Verification items for the finished model (mm, model axes). Face numbers are marked on the shaded views. A direction names the side the tool comes from. Give positions to 0.01 mm unless a question says otherwise; leave off trailing zeros. Loops run counter-clockwise (first coordinate to the right, second up) from the corner with the lowest first, then second, coordinate; pieces in that order, holes last. Notation, with made-up numbers: (72, 56.5) -> (131, 56.5) arc R33 ccw to (131, 91.5) -> close; hole circle Ø7 at (85, -12). An arc over 180 degrees is marked (long way). Answer in a Markdown table with one row per item. Add a question column.
Q1. Set-up check for the marked faces 1 and 2: record each of +Z, -Z, +X, -X, +Y, -Y from which the full face is reachable in a straight line by a thin tool's end or side.
Q2. Section check A-A on y = 3.5. Enter the section's corners in (x, z).
Q3. Gauge pin test, flat ends, axial feed: P1, Ø3, axis at x = 19, z = -11.5, coming from the +Y side; P2, Ø2, axis at x = 19, z = 6.5, coming from the -Y side (3 decimals); P3, Ø2, axis at x = 20, y = -6.5, coming from the -Z side (3 decimals). Record the tip position at first contact, or that the pin passes through.
Q4. Section check C-C on x = 17. Enter the section's corners in (y, z), and give its area (3 significant figures).
Q5. Section check B-B on z = -4. Enter the section's corners in (x, y).
Q6. Section check D-D on z = -13.5. Enter the section's corners in (x, y).
Q7. Material ranges on probe 1 along Y at (x, z) = (15, 0); probe 2 along Y at (x, z) = (18.25, 7); probe 3 along Z at (x, y) = (17.75, -7.5), recorded low to high.
Q8. Release check for a two-part mould opening along Y. For the marked faces 3, 4 and 5 record: pulls with the +Y half, pulls with the -Y half, needs draft (parallel to the pull), parting line crosses it, or undercut.
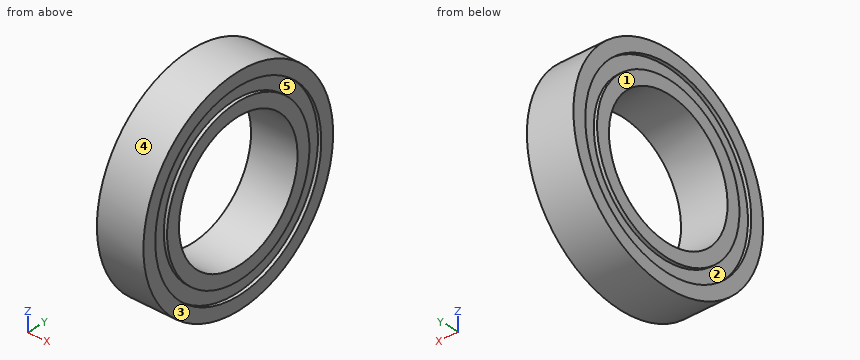
```python
from build123d import *


with BuildPart() as part:
    # Sketch1 → Revolve1 (revolve)
    with BuildSketch(Plane.XY, mode=Mode.PRIVATE) as revolve1_sk:
        Polygon((14.644406169, 14), (14.644406169, 16), (21.644406169, 16), (21.644406169, 14), (21.144406169, 14), (21.144406169, 12), (21.644406169, 12), (21.644406169, 10), (14.644406169, 10), (14.644406169, 12), (15.144406169, 12), (15.144406169, 14), align=None)
    revolve(revolve1_sk.sketch.rotate(Axis((0, 0, 0), (1, 0, 0)), 90), axis=Axis((0, 0, 0), (1, 0, 0)))


solid = part.part
```
Taken from the geometry:
| question | item | result |
|---|---|---|
| 1 | face 1 | +Z, -Z, -X, +Y, -Y |
| 1 | face 2 | -X |
| 2 | outline | (14.64, -15.61) -> (21.64, -15.61) -> (21.64, -13.56) -> (21.14, -13.56) -> (21.14, -11.48) -> (21.64, -11.48) -> (21.64, -9.37) -> (14.64, -9.37) -> (14.64, -11.48) -> (15.14, -11.48) -> (15.14, -13.56) -> (14.64, -13.56) -> close; (14.64, 9.37) -> (21.64, 9.37) -> (21.64, 11.48) -> (21.14, 11.48) -> (21.14, 13.56) -> (21.64, 13.56) -> (21.64, 15.61) -> (14.64, 15.61) -> (14.64, 13.56) -> (15.14, 13.56) -> (15.14, 11.48) -> (14.64, 11.48) -> close |
| 3 | P1 | stops at y = 12.49 |
| 3 | P2 | stops at y = -15.025 |
| 3 | P3 | stops at z = -15.025 |
| 4 | outline | circle Ø32 at (0, 0); hole circle Ø20 at (0, 0) |
| 4 | area | 490 mm² |
| 5 | outline | (14.64, -15.49) -> (21.64, -15.49) -> (21.64, -13.42) -> (21.14, -13.42) -> (21.14, -11.31) -> (21.64, -11.31) -> (21.64, -9.17) -> (14.64, -9.17) -> (14.64, -11.31) -> (15.14, -11.31) -> (15.14, -13.42) -> (14.64, -13.42) -> close; (14.64, 9.17) -> (21.64, 9.17) -> (21.64, 11.31) -> (21.14, 11.31) -> (21.14, 13.42) -> (21.64, 13.42) -> (21.64, 15.49) -> (14.64, 15.49) -> (14.64, 13.42) -> (15.14, 13.42) -> (15.14, 11.31) -> (14.64, 11.31) -> close |
| 6 | outline | (14.64, -8.59) -> (21.64, -8.59) -> (21.64, -3.71) -> (21.14, -3.71) -> (21.14, 3.71) -> (21.64, 3.71) -> (21.64, 8.59) -> (14.64, 8.59) -> (14.64, 3.71) -> (15.14, 3.71) -> (15.14, -3.71) -> (14.64, -3.71) -> close |
| 7 | probe 1 | y = -16 to -14, -12 to -10, 10 to 12, 14 to 16 |
| 7 | probe 2 | y = -14.39 to -7.14, 7.14 to 14.39 |
| 7 | probe 3 | z = -14.13 to -6.61, 6.61 to 14.13 |
| 8 | face 3 | needs draft |
| 8 | face 4 | parting line crosses it |
| 8 | face 5 | undercut |
